```python
from build123d import *

# Parameters (mm, degrees)
SKETCH1_R           = 1.5
BOSS_EXTRUDE1_DEPTH = 2


with BuildPart() as part:
    # Sketch1 → Boss-Extrude1 (new body)
    with BuildSketch(Plane.XY):
        with BuildLine():
            Line((-10.160254038, 2.401923789), (7.160254038, -7.598076211))
            ThreePointArc((7.160254038, -7.598076211), (11.258330249, -6.5), (10.160254038, -2.401923789))
            Line((10.160254038, -2.401923789), (-7.160254038, 7.598076211))
            ThreePointArc((-7.160254038, 7.598076211), (-11.258330249, 6.5), (-10.160254038, 2.401923789))
        make_face()
        Circle(SKETCH1_R, mode=Mode.SUBTRACT)
        with Locations((8.660254038, -5)):
            Circle(SKETCH1_R, mode=Mode.SUBTRACT)
        with Locations((-8.660254038, 5)):
            Circle(SKETCH1_R, mode=Mode.SUBTRACT)
    extrude(amount=BOSS_EXTRUDE1_DEPTH)


solid = part.part
```
Part model, mm, in its own coordinate system. Give positions to 0.01 mm unless a question says otherwise; leave off trailing zeros. Write each loop counter-clockwise with the first axis right and the second up, starting at its lowest first coordinate (ties: lowest second). Pieces come first, ordered by that corner, then holes. Notation, with made-up numbers: M 75,41 L 85,41 A13 cw 85,52 Z; hole C -32,-11.5 d8. An arc over 180 degrees is marked long. Use CSV: the item, a comma, the result in double quotes.
Item 1: Slice it at C-C on x = 0. Write the cut outline in (y, z).
Taken from the geometry:
outline,"M -3.46,0 L -1.5,0 L -1.5,2 L -3.46,2 Z; M 1.5,0 L 3.46,0 L 3.46,2 L 1.5,2 Z"
Item 2: Slice it at B-B on z = 1.6. Write the cut outline in (x, y), plus the area to 3 significant figures.
Taken from the geometry:
outline,"M -10.16,2.4 L 7.16,-7.6 A3 ccw 10.16,-2.4 L -7.16,7.6 A3 ccw Z; hole C -8.66,5 d3; hole C 0,0 d3; hole C 8.66,-5 d3"
area,"127 mm²"
Item 3: Pull direction Y, two halves, no side cores. Call faces 1 (the face through (-11.2, 6.6, 1)), 2 (the face through (-1.5, 0.07, 0.99)), 3 (the face through (-1.62, -2.53, 0.99)), 4 (the face through (8.465, -3.513, 0.986)): +Y half, -Y half, draft (parallel to the pull), parting line (faces both ways), or undercut.
Taken from the geometry:
face 1,"parting line"
face 2,"undercut"
face 3,"-Y half"
face 4,"undercut"
Item 4: Slice it at D-D on x = 4.5. Write the cut outline in (y, z).
Taken from the geometry:
outline,"M -6.06,0 L 0.87,0 L 0.87,2 L -6.06,2 Z"
Item 5: Slice it at A-A on y = 0. Write the cut outline in (x, z), plus the area to 3 significant figures.
Taken from the geometry:
outline,"M -6,0 L -1.5,0 L -1.5,2 L -6,2 Z; M 1.5,0 L 6,0 L 6,2 L 1.5,2 Z"
area,"18.0 mm²"
Item 6: Drill centre lines: probe 1 along Y at (x, z) = (9, 1.9); probe 2 along X at (y, z) = (5.25, 1.7); probe 3 along Y at (x, z) = (-0.5, 0.8). Where is each one in solid material? Low to high.
Taken from the geometry:
probe 1,"y = -7.98 to -6.46, -3.54 to -1.73"
probe 2,"x = -11.65 to -10.14, -7.18 to -3.09"
probe 3,"y = -3.18 to -1.41, 1.41 to 3.75"
